Input: part model. Units: mm. Frame: model coordinates. A direction names the side the tool comes from. Coordinates: 2 decimals unless noted, no trailing zeros. Loops run counter-clockwise (first coordinate to the right, second up) from the corner with the lowest first, then second, coordinate; pieces in that order, holes last.
```python
from build123d import *

# Parameters (mm, degrees)
SKETCH_1_W          = 30
SKETCH_1_H          = 20
EXTRUDE_1_DEPTH     = 5
SKETCH_2_W          = 5
SKETCH_2_H          = 20
EXTRUDE_2_DEPTH     = 5
SKETCH_4_W          = 35
SKETCH_4_H          = 10
CUT_EXTRUDE_1_DEPTH = 1
SKETCH_5_W          = 20
SKETCH_5_H          = 20
EXTRUDE_4_DEPTH     = 5
CHAMFER_1_SIZE      = 3
CHAMFER_2_SIZE      = 3
M3X0_5_1_D          = 2.5
MOVE_FACE_1_BY      = 3


with BuildPart() as part:
    # 草图1 → 凸台-拉伸1 (new body)
    with BuildSketch(Plane.XY):
        Rectangle(SKETCH_1_W, SKETCH_1_H)
    extrude(amount=EXTRUDE_1_DEPTH)

    # 草图2 → 凸台-拉伸2 (add)
    with BuildSketch(Plane(origin=(15, 0, 0), x_dir=(0, 0, -1), z_dir=(1, 0, 0))):
        with Locations((-2.5, 0)):
            Rectangle(SKETCH_2_W, SKETCH_2_H)
    extrude(amount=EXTRUDE_2_DEPTH)

    # 草图4 → 切除-拉伸1 (cut)
    with BuildSketch(Plane(origin=(0, 0, 0), x_dir=(-1, 0, 0), z_dir=(0, 0, -1))):
        with Locations((-2.5, 0)):
            Rectangle(SKETCH_4_W, SKETCH_4_H)
    extrude(amount=-CUT_EXTRUDE_1_DEPTH, mode=Mode.SUBTRACT)

    # 草图5 → 凸台-拉伸4 (add)
    with BuildSketch(Plane.XY.offset(5)):
        with Locations((24, 0)):
            Rectangle(SKETCH_5_W, SKETCH_5_H)
    extrude(amount=EXTRUDE_4_DEPTH)

    # 倒角1
    chamfer_1_edges = [part.edges().sort_by_distance(p)[0] for p in [
        (14, 0, 10),
    ]]
    chamfer(chamfer_1_edges, length=CHAMFER_1_SIZE)

    # 倒角2
    chamfer_2_edges = [part.edges().sort_by_distance(p)[0] for p in [
        (34, 0, 10),
    ]]
    chamfer(chamfer_2_edges, length=CHAMFER_2_SIZE)

    # M3x0.5 螺纹孔1 (through all)
    with Locations(Plane.XY.offset(5)):
        with Locations((-10, 0), (-1, 0)):
            Hole(M3X0_5_1_D / 2)

    # Move Face 1: a face moved outward by 3.0
    extrude(part.faces().sort_by_distance((27, 0, 5))[0], amount=MOVE_FACE_1_BY, dir=(0, 0, -1))


solid = part.part
```
Item 1: Reachability of faces 4 (the face through (20, 0.1, 1.2)), 5 (the face through (-1, 2, 5)), 6 (the face through (2.7, 5, 0.5)) from +Z, -Z, +X, -X, +Y, -Y: full face, straight path, thin tool, end or side. Return the list, or none.
Result:
face 4: -Z, +X, +Y, -Y
face 5: +Z, -X, +Y, -Y
face 6: -Z, +X, -X
Item 2: Contact query for flat-ended pins moving along their axis: P1, Ø6, axis at x = -9.5, z = 8.5, coming from the +Y side; P2, Ø11, axis at x = 24, y = 0.5, coming from the -Z side; P3, Ø1, axis at y = -2.5, z = 6.5, coming from the -X side; P4, Ø2, axis at x = 25, y = -5, coming from the -Z side. Output: stop coordinate, or through.
Result:
P1: passes through
P2: stops at z = 1
P3: stops at x = 14
P4: stops at z = 2
Item 3: Section query A-A (y = 0). Output: boundary loops of the cut face in (x, z), then the cut area to 3 significant figures.
Result:
outline: (-15, 1) - (-11.25, 1) - (-11.25, 5) - (-15, 5) - close; (-8.75, 1) - (-2.25, 1) - (-2.25, 5) - (-8.75, 5) - close; (0.25, 1) - (20, 1) - (20, 2) - (34, 2) - (34, 7) - (31, 10) - (17, 10) - (14, 7) - (14, 5) - (0.25, 5) - close
area: 253 mm2
Item 4: Mould query, pull axis Y, two halves, no side actions, for faces 1 (the face through (3, 0, 1)), 2 (the face through (24, 0, 10)), 3 (the face through (15, 10, 4)). Classes: +Y half, -Y half, draft (parallel to the pull), parting line (faces both ways), or undercut.
Result:
face 1: undercut
face 2: draft
face 3: +Y half
Item 5: Section query D-D (x = 9.5). Output: boundary loops of the cut face in (y, z).
Result:
outline: (-10, 0) - (-5, 0) - (-5, 1) - (5, 1) - (5, 0) - (10, 0) - (10, 5) - (-10, 5) - close
Item 6: Section query C-C (y = -2.25). Output: boundary loops of the cut face in (x, z), then the cut area to 3 significant figures.
Result:
outline: (-15, 1) - (20, 1) - (20, 2) - (34, 2) - (34, 7) - (31, 10) - (17, 10) - (14, 7) - (14, 5) - (-15, 5) - close
area: 273 mm2
Item 7: Line query: L1, parallel to X at y = -0.5, z = 4.75; L2, parallel to Y at x = -1, z = 2.3; L3, parallel to X at y = 4.5, z = 6. Output: solid intervals per line, ascending.
Result:
L1: x = -15 to -11.15, -8.85 to -2.15, 0.15 to 34
L2: y = -10 to -1.25, 1.25 to 10
L3: x = 14 to 34
Item 8: Section query B-B (x = -1). Output: boundary loops of the cut face in (y, z).
Result:
outline: (-10, 0) - (-5, 0) - (-5, 1) - (-1.25, 1) - (-1.25, 5) - (-10, 5) - close; (1.25, 1) - (5, 1) - (5, 0) - (10, 0) - (10, 5) - (1.25, 5) - close
